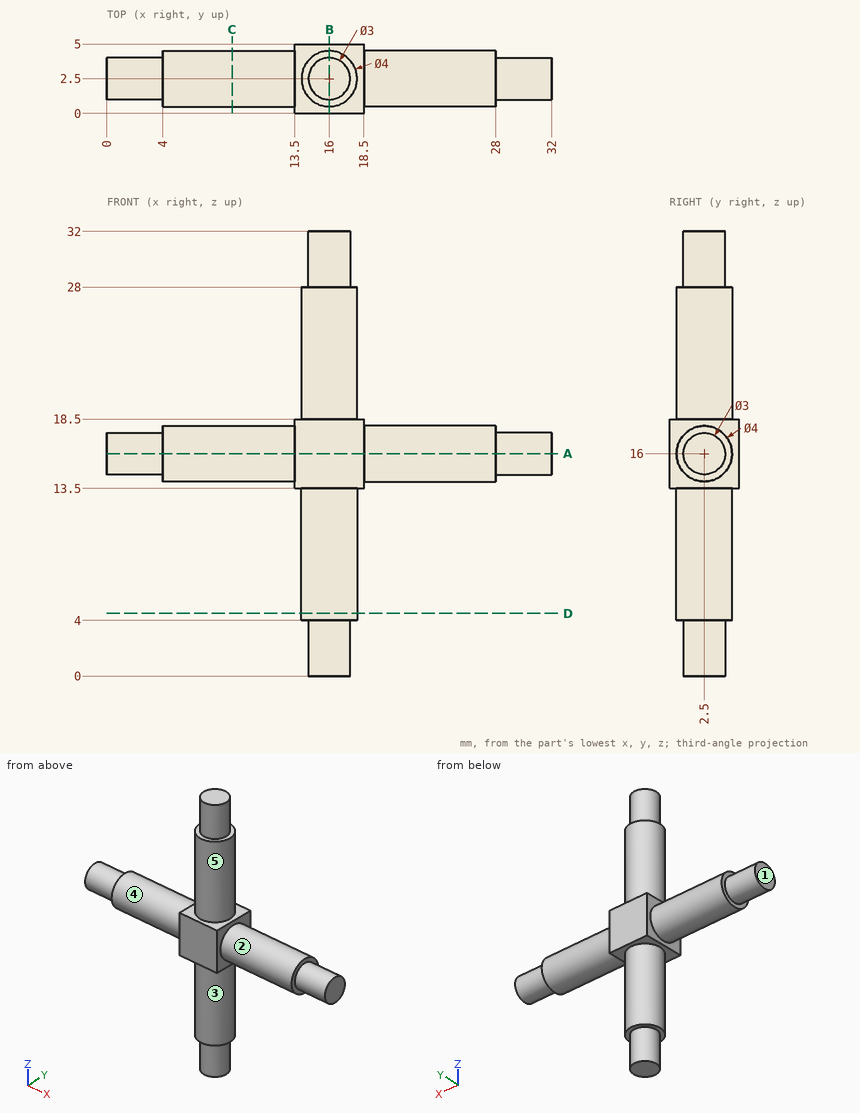
Design review of the part shown in the three views and the two pictorial views. Dimensions are in mm from the part's minimum x, y and z. A direction names the side the tool comes from. Round coordinates to 2 decimals unless told otherwise and drop trailing zeros. Order: outer loops, then holes, each group sorted by start corner. A loop starts at its lowest first (then second) coordinate and runs counter-clockwise, first axis right, second up.
(1) Take a section at C-C, the plane x = 9. State the section outline as (y, z) points, plus the area to 3 significant figures.
Working result:
outline: circle Ø4 at (2.5, 16)
area: 12.6 mm2
(2) Take a section at D-D, the plane z = 4.5. State the section outline as (x, y) points.
Working result:
outline: circle Ø4 at (16, 2.5)
(3) Take a section at B-B, the plane x = 16. State the section outline as (y, z) points, plus the area to 3 significant figures.
Working result:
outline: (0, 13.5) - (0.5, 13.5) - (0.5, 4) - (1, 4) - (1, 0) - (4, 0) - (4, 4) - (4.5, 4) - (4.5, 13.5) - (5, 13.5) - (5, 18.5) - (4.5, 18.5) - (4.5, 28) - (4, 28) - (4, 32) - (1, 32) - (1, 28) - (0.5, 28) - (0.5, 18.5) - (0, 18.5) - close
area: 125 mm2
(4) Tool access review of the marked faces 1, 2, 3, 4 and 5: name each direction out of +Z, -Z, +X, -X, +Y, -Y from which nothing blocks a thin tool from reaching the whole face with its end or side.
Working result:
face 1: +Z, -Z, -X, +Y, -Y
face 2: +X
face 3: -Z
face 4: -X
face 5: +Z
(5) Wall thickness on L1, parallel to Z at x = 16, y = 0.6; L2, parallel to X at y = 2.35, z = 8; L3, parallel to Z at x = 17, y = 4.55: over which ranges is each line inside the solid? List them lowest first.
Working result:
L1: z = 4 to 28
L2: x = 14.01 to 17.99
L3: z = 13.5 to 18.5
(6) Take a section at A-A, the plane z = 16. State the section outline as (x, y) points.
Working result:
outline: (0, 1) - (4, 1) - (4, 0.5) - (13.5, 0.5) - (13.5, 0) - (18.5, 0) - (18.5, 0.5) - (28, 0.5) - (28, 1) - (32, 1) - (32, 4) - (28, 4) - (28, 4.5) - (18.5, 4.5) - (18.5, 5) - (13.5, 5) - (13.5, 4.5) - (4, 4.5) - (4, 4) - (0, 4) - close
(7) For P1, Ø2, axis at x = 18, y = 1.5, coming from the -Z side; P2, Ø1.5, axis at x = 4, y = 3, coming from the -Z side; P3, Ø3, axis at y = 1, z = 6, coming from the -X side, all flat-tipped, find the tip position at first contact; note any pin that passes through.
Working result:
P1: stops at z = 0
P2: stops at z = 14
P3: stops at x = 14
